Build history of the part. All positions in model axes, mm. A direction names the side the tool comes from. Coordinates: 2 decimals unless noted, no trailing zeros. Write each loop counter-clockwise with the first axis right and the second up, starting at its lowest first coordinate (ties: lowest second). Pieces come first, ordered by that corner, then holes. Notation, with made-up numbers: (-23.75, 1.25) -> (-19.75, 1.25) arc R24 ccw to (-19.75, 16.25) -> close; hole circle Ø5 at (40, 26). An arc over 180 degrees is marked (long way). Write each question's results on one line, items separated by ' | '. Start each with the question number.
Q1. Saw through at A-A on x = 155.5. Give the cut face in (y, z), and give its area (3 significant figures).
Q2. Drop flat-ended pins along their axis: pin 1 Ø1.5 at (x, z) = (-5, -1.5) entering from +Y; pin 2 Ø1.5 at (x, z) = (167, 1) entering from +Y; pin 3 Ø1.5 at (x, y) = (-45, 3) entering from +Z. Give the stop position or say it passes through.
Q3. Tool access for faces 5 (the face through (3, -4.88, 1.08)), 6 (the face through (215, -2, -2)): list every direction of +Z, -Z, +X, -X, +Y, -Y with a clear straight run to the whole face (end or side of a thin tool).
Q4. Drill centre lines: line 1 (X direction, y = -1.5, z = -2.25); line 2 (Y direction, x = 197.5, z = -3); line 3 (Z direction, x = -69, y = -2.25). Where is each one in solid material? Low to high.
Q5. Two-plate mould, pull along X, no slides. Class faces 1 (the face through (-215, 0, 0)), 2 (the face through (217, 2, -2)), 3 (the face through (219.218, -3.905, 0.867)), 4 (the face through (222, 0, 0)): released by +X, released by -X, zero draft, split by the parting line, or undercut.
from build123d import *

# Parameters (mm, degrees)
SKETCH1_R           = 5
BOSS_EXTRUDE1_DEPTH = 215
SKETCH2_R           = 2.5
BOSS_EXTRUDE2_DEPTH = 2
SKETCH3_R           = 4
BOSS_EXTRUDE3_DEPTH = 5
CHAMFER1_SIZE       = 0.5


with BuildPart() as part:
    # Sketch1 → Boss-Extrude1 (new, symmetric)
    with BuildSketch(Plane(origin=(0, 0, 0), x_dir=(0, 0, -1), z_dir=(1, 0, 0))):
        Circle(SKETCH1_R)
    extrude(amount=BOSS_EXTRUDE1_DEPTH, both=True)

    # Sketch2 → Boss-Extrude2 (add)
    with BuildSketch(Plane(origin=(215, 0, 0), x_dir=(0, 0, -1), z_dir=(1, 0, 0))):
        Circle(SKETCH2_R)
    extrude(amount=BOSS_EXTRUDE2_DEPTH)

    # Sketch3 → Boss-Extrude3 (add)
    with BuildSketch(Plane(origin=(217, 0, 0), x_dir=(0, 0, -1), z_dir=(1, 0, 0))):
        Circle(SKETCH3_R)
    extrude(amount=BOSS_EXTRUDE3_DEPTH)

    # Chamfer1
    chamfer1_edges = [part.edges().sort_by_distance(p)[0] for p in [
        (-215, 0, 5),
        (215, 0, 5),
        (222, 0, 4),
    ]]
    chamfer(chamfer1_edges, length=CHAMFER1_SIZE)


solid = part.part
Returned:
1) outline: circle Ø10 at (0, 0) | area: 78.5 mm2
2) pin 1: stops at y = 4.94 | pin 2: stops at y = 4.99 | pin 3: stops at z = 4.47
3) face 5: +X, -X | face 6: none
4) line 1: x = -215 to 215, 217 to 222 | line 2: y = -4 to 4 | line 3: z = -4.47 to 4.47
5) face 1: released by -X | face 2: undercut | face 3: zero draft | face 4: released by +X
